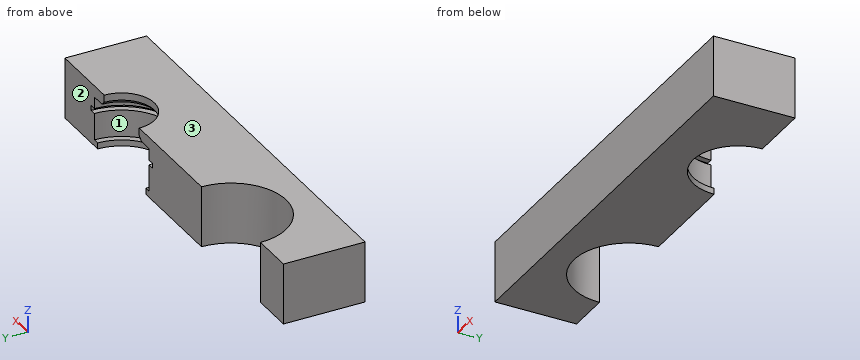
```python
from build123d import *

# Parameters (mm, degrees)
SKETCH1_W               = 1000
SKETCH1_H               = 200
BOSS_EXTRUDE1_DEPTH     = 150
CUT_EXTRUDE1_DEPTH      = 1031.776406404
CUT_EXTRUDE1_DEPTH_BACK = 1031.776406404
SKETCH2_R               = 135
SKETCH2_R_2             = 80
CHAMFER1_SIZE           = 10


with BuildPart() as part:
    # Sketch1 → Boss-Extrude1 (new body)
    with BuildSketch(Plane.XY):
        with Locations((500, -100)):
            Rectangle(SKETCH1_W, SKETCH1_H)
    extrude(amount=BOSS_EXTRUDE1_DEPTH)

    # Sketch2 → Cut-Extrude1 (cut, two sides: drawn at the far end of the back side and taken through both)
    with BuildSketch(Plane.XY.offset(150).offset(-CUT_EXTRUDE1_DEPTH_BACK)):
        with Locations((240, 0)):
            Circle(SKETCH2_R)
        with Locations((740, 0)):
            Circle(SKETCH2_R_2)
    extrude(amount=CUT_EXTRUDE1_DEPTH + CUT_EXTRUDE1_DEPTH_BACK, mode=Mode.SUBTRACT)

    # Sketch3 → Cut-Revolve1 (revolve, cut)
    with BuildSketch(Plane(origin=(0, 0, 0), x_dir=(1, 0, 0), z_dir=(0, 1, 0))):
        Polygon((740, -150), (660, -150), (660, -122), (615, -122), (615, -93), (600, -93), (600, -81), (615, -81), (615, -15), (630, -15), (630, 0), (740, 0), align=None)
    revolve(axis=Axis((740, 0, 0), (0, 0, 1)), mode=Mode.SUBTRACT)

    # Chamfer1
    chamfer1_edges = [part.edges().sort_by_distance(p)[0] for p in [
        (740, -80, 122),
    ]]
    chamfer(chamfer1_edges, length=CHAMFER1_SIZE)


solid = part.part
```
Design review of the part built by this model. Coordinates are the model's own, in mm. Face numbers are marked on the shaded views. Round coordinates to 2 decimals unless told otherwise and drop trailing zeros. Order: outer loops, then holes, each group sorted by start corner. A loop starts at its lowest first (then second) coordinate and runs counter-clockwise, first axis right, second up. Notation, with made-up numbers: M 27,-19.75 L 49,-19.75 A27 ccw 49,17.25 Z; hole C 75.5,89 d4. An arc over 180 degrees is marked long. Put each result on its own line as item: value.
Q1. To check wall thickness, follow line 1 (X direction, y = -69.5, z = 126); line 2 (X direction, y = -59, z = 36.5); line 3 (Y direction, x = 786.5, z = 30). State the ranges of each line that lie inside material, in increasing order.
Reported:
line 1: 0 to 124.26, 355.74 to 689.35, 790.65 to 1000
line 2: 0 to 118.58, 361.42 to 629.8, 850.2 to 1000
line 3: -200 to -116.03
Q2. Consider section C-C (y = -21.5). State how many separate pieces and enclosed holes the cut face has, and give its area (3 significant figures).
Reported:
separate pieces: 3
enclosed holes: 0
area: 75,600 mm²
Q3. Draft analysis for pull direction Z (two halves, no side actions). For the marked faces 1, 2 and 3, state which applies: released by +Z, released by -Z, zero draft, split by the parting line, or undercut.
Reported:
face 1: undercut
face 2: zero draft
face 3: released by +Z
Q4. Consider section D-D (x = 240). State the section outline as (y, z) points, and give its area (3 significant figures).
Reported:
outline: M -200,0 L -135,0 L -135,150 L -200,150 Z
area: 9,750 mm²
Q5. Consider section A-A (x = 740). State the section outline as (y, z) points, and give its area (3 significant figures).
Reported:
outline: M -200,0 L -110,0 L -110,15 L -125,15 L -125,81 L -140,81 L -140,93 L -125,93 L -125,122 L -90,122 L -80,132 L -80,150 L -200,150 Z
area: 12,500 mm²
Q6. Consider section B-B (z = 25.5). State the section outline as (x, y) points.
Reported:
outline: M 0,-200 L 1000,-200 L 1000,0 L 865,0 A125 cw 615,0 L 375,0 A135 cw 105,0 L 0,0 Z
Q7. Insertion check: pin 1 Ø6 at (x, z) = (255.5, 101.5) entering from +Y; pin 2 Ø3 at (x, z) = (770, 130) entering from +Y; pin 3 Ø8 at (x, z) = (138, 24) entering from +Y. Each pin has a flat end and moves straight along its axis. Give the tip position at first contact, or say it passes through.
Reported:
pin 1: y = -133.73
pin 2: y = -74.59
pin 3: y = -83.6
